```python
from build123d import *

# Parameters (mm, degrees)
SKETCH1_W               = 64
SKETCH1_H               = 48
BOSS_EXTRUDE1_DEPTH     = 4
CUT_EXTRUDE1_DEPTH      = 41.199502484
CUT_EXTRUDE1_DEPTH_BACK = 41.199502484
SKETCH2_R               = 1.5


with BuildPart() as part:
    # Sketch1 → Boss-Extrude1 (new body)
    with BuildSketch(Plane.XY):
        Rectangle(SKETCH1_W, SKETCH1_H)
    extrude(amount=BOSS_EXTRUDE1_DEPTH)

    # Sketch2 → Cut-Extrude1 (cut, two sides: drawn at the far end of the back side and taken through both)
    with BuildSketch(Plane.XY.offset(4).offset(-CUT_EXTRUDE1_DEPTH_BACK)):
        with Locations((28.95, -20.95)):
            Circle(SKETCH2_R)
        with Locations(Location((-28.95, -20.95, 0), (0, 0, 180))):
            Circle(SKETCH2_R)
        with Locations(Location((28.95, 20.95, 0), (0, 0, 180))):
            Circle(SKETCH2_R)
        with Locations((-28.95, 20.95)):
            Circle(SKETCH2_R)
    extrude(amount=CUT_EXTRUDE1_DEPTH + CUT_EXTRUDE1_DEPTH_BACK, mode=Mode.SUBTRACT)


solid = part.part
```
Model file for the job. Use its own axes, mm. Round coordinates to 2 decimals unless told otherwise and drop trailing zeros. Write each loop counter-clockwise with the first axis right and the second up, starting at its lowest first coordinate (ties: lowest second). Pieces come first, ordered by that corner, then holes. Notation, with made-up numbers: (78, 76.25) -> (122, 76.25) arc R27 cw to (122, 110.25) -> close; hole circle Ø9 at (-8.5, 56). An arc over 180 degrees is marked (long way). Answer as CSV lines item,"result".
1. Drill centre lines: line 1 (Y direction, x = -28.95, z = 2.9); line 2 (X direction, y = 21.5, z = 0.35). Where is each one in solid material? Low to high.
Resolved:
line 1,"-24 to -22.45, -19.45 to 19.45, 22.45 to 24"
line 2,"-32 to -30.35, -27.55 to 27.55, 30.35 to 32"
2. Pin check, flat tip, straight feed: pin 1 Ø6 at (x, y) = (11.5, -17) entering from -Z. Stop position of the tip, or through.
Resolved:
pin 1,"z = 0"
3. Slice it at B-B, the plane y = -20.95. List the corners of the cut face in (x, z).
Resolved:
outline,"(-32, 0) -> (-30.45, 0) -> (-30.45, 4) -> (-32, 4) -> close; (-27.45, 0) -> (27.45, 0) -> (27.45, 4) -> (-27.45, 4) -> close; (30.45, 0) -> (32, 0) -> (32, 4) -> (30.45, 4) -> close"
4. Slice it at A-A, the plane x = -28.95. List the corners of the cut face in (y, z), plus the area to 3 significant figures.
Resolved:
outline,"(-24, 0) -> (-22.45, 0) -> (-22.45, 4) -> (-24, 4) -> close; (-19.45, 0) -> (19.45, 0) -> (19.45, 4) -> (-19.45, 4) -> close; (22.45, 0) -> (24, 0) -> (24, 4) -> (22.45, 4) -> close"
area,"168 mm²"
5. Mould opens along X. For faces 1 (the face through (28.3, 22.3, 2)), 2 (the face through (0, -24, 2)), 3 (the face through (32, 0, 2)), 4 (the face through (-32, 0, 2)) say: +X half, -X half, draft (parallel to the pull), parting line (faces both ways), or undercut.
Resolved:
face 1,"undercut"
face 2,"draft"
face 3,"+X half"
face 4,"-X half"
